from build123d import *

# Parameters (mm, degrees)
EXTRUDE_1_DEPTH     = 100
SKETCH_2_W          = 35.317953013
SKETCH_2_H          = 4.2
CUT_EXTRUDE_1_DEPTH = 60


with BuildPart() as part:
    # 草图1 → 凸台-拉伸1 (new body)
    with BuildSketch(Plane.XY):
        Polygon((-37.5, 32.788461538), (42.5, 32.788461538), (42.5, 22.788461538), (-27.5, 22.788461538), (-27.5, -37.211538462), (-37.5, -37.211538462), align=None)
    extrude(amount=EXTRUDE_1_DEPTH)

    # 草图2 → 切除-拉伸1 (cut)
    with BuildSketch(Plane.XY.offset(100)):
        with Locations((-12.799064643, 30.688461538)):
            Rectangle(SKETCH_2_W, SKETCH_2_H)
    extrude(amount=-CUT_EXTRUDE_1_DEPTH, mode=Mode.SUBTRACT)


solid = part.part
Can you work these out from the model? Positions are in its coordinate system, mm. A direction names the side the tool comes from. Coordinates: 2 decimals unless noted, no trailing zeros. Write each loop counter-clockwise with the first axis right and the second up, starting at its lowest first coordinate (ties: lowest second). Pieces come first, ordered by that corner, then holes.
Q1. Please list where these lines run through material, in increasing order: L1, parallel to X at y = 29, z = 58; L2, parallel to X at y = 16, z = 90; L3, parallel to Y at x = 0.5, z = 39.
Results found:
L1: x = -37.5 to -30.46, 4.86 to 42.5
L2: x = -37.5 to -27.5
L3: y = 22.79 to 32.79
Q2. Imagine slicing it at B-B, the plane x = 16.5. List the corners of the cut face in (y, z) for me.
Results found:
outline: (22.79, 0) - (32.79, 0) - (32.79, 100) - (22.79, 100) - close
Q3. Imagine slicing it at A-A, the plane z = 42. List the corners of the cut face in (x, y) for me.
Results found:
outline: (-37.5, -37.21) - (-27.5, -37.21) - (-27.5, 22.79) - (42.5, 22.79) - (42.5, 32.79) - (4.86, 32.79) - (4.86, 28.59) - (-30.46, 28.59) - (-30.46, 32.79) - (-37.5, 32.79) - close
Q4. Which directions (+Z, -Z, +X, -X, +Y, -Y) give clear straight access to the entire face, cutting with the end or side of a thin tool? Please do faces 1 (the face through (-6, 24, 100)), 2 (the face through (-13, 31, 40)), 3 (the face through (8, 22.788, 49)).
Results found:
face 1: +Z, +X, -X, +Y, -Y
face 2: +Z, +Y
face 3: +Z, -Z, +X, -Y
Q5. Imagine slicing it at D-D, the plane z = 8. List the corners of the cut face in (x, y) for me.
Results found:
outline: (-37.5, -37.21) - (-27.5, -37.21) - (-27.5, 22.79) - (42.5, 22.79) - (42.5, 32.79) - (-37.5, 32.79) - close
Q6. For P1, Ø4.5, axis at x = -15.5, y = 31.5, coming from the +Z side; P2, Ø4, axis at x = 34, z = 13.5, coming from the -Y side; P3, Ø8, axis at x = -12.5, z = 87.5, coming from the +Y side, each with a flat end and sliding along its axis, tell me the tip position at first contact or that it passes through.
Results found:
P1: stops at z = 40
P2: stops at y = 22.79
P3: stops at y = 28.59
Q7. Imagine slicing it at C-C, the plane y = -2. List the corners of the cut face in (x, z) for me.
Results found:
outline: (-37.5, 0) - (-27.5, 0) - (-27.5, 100) - (-37.5, 100) - close
